from build123d import *

# Parameters (mm, degrees)
SKETCH3_R           = 46
SKETCH3_R_2         = 40
BOSS_EXTRUDE1_DEPTH = 215
SKETCH4_R           = 160
CUT_EXTRUDE1_DEPTH  = 900
CUT_EXTRUDE2_START  = -300
SKETCH5_R           = 40
CUT_EXTRUDE2_DEPTH  = 300
SKETCH6_R           = 67.5
SKETCH6_R_2         = 40
BOSS_EXTRUDE2_DEPTH = 15


with BuildPart() as part:
    # Sketch1 → Revolve1 (revolve)
    with BuildSketch(Plane.XY, mode=Mode.PRIVATE) as revolve1_sk:
        Polygon((0, 160), (0, 215), (40, 215), (40, 180), (1360, 180), (1390, 150), (1520, 150), (1520, 180), (1580, 180), (1580, 130), (1381.715728753, 130), (1351.715728753, 160), align=None)
    revolve(revolve1_sk.sketch.rotate(Axis((0, 0, 0), (1, 0, 0)), 90), axis=Axis((0, 0, 0), (1, 0, 0)))

    # Sketch3 → Boss-Extrude1 (add)
    with BuildSketch(Plane(origin=(0, 0, 0), x_dir=(1, 0, 0), z_dir=(0, 1, 0))):
        with Locations(Location((380, 0, 0), (0, 0, 90))):
            Circle(SKETCH3_R)
        with Locations(Location((380, 0, 0), (0, 0, 90))):
            Circle(SKETCH3_R_2, mode=Mode.SUBTRACT)
    extrude(amount=BOSS_EXTRUDE1_DEPTH)

    # Sketch4 → Cut-Extrude1 (cut)
    with BuildSketch(Plane.ZY):
        Circle(SKETCH4_R)
    extrude(amount=-CUT_EXTRUDE1_DEPTH, mode=Mode.SUBTRACT)

    # Sketch5 → Cut-Extrude2 (cut)
    with BuildSketch(Plane(origin=(0, 215, 0), x_dir=(1, 0, 0), z_dir=(0, 1, 0)).offset(CUT_EXTRUDE2_START)):
        with Locations(Location((380, 0, 0), (0, 0, 270))):
            Circle(SKETCH5_R)
    extrude(amount=CUT_EXTRUDE2_DEPTH, mode=Mode.SUBTRACT)

    # Sketch6 → Boss-Extrude2 (add)
    with BuildSketch(Plane(origin=(0, 215, 0), x_dir=(1, 0, 0), z_dir=(0, 1, 0))):
        with Locations(Location((380, 0, 0), (0, 0, 270))):
            Circle(SKETCH6_R)
        with Locations(Location((380, 0, 0), (0, 0, 270))):
            Circle(SKETCH6_R_2, mode=Mode.SUBTRACT)
    extrude(amount=BOSS_EXTRUDE2_DEPTH)


solid = part.part
Verification items for the finished model (mm, model axes). A direction names the side the tool comes from. Coordinates: 2 decimals unless noted, no trailing zeros. Write each loop counter-clockwise with the first axis right and the second up, starting at its lowest first coordinate (ties: lowest second). Pieces come first, ordered by that corner, then holes. Notation, with made-up numbers: M 60.5,-13.5 L 95.5,-13.5 A18 cw 95.5,13.5 Z; hole C 0.5,80.5 d5. An arc over 180 degrees is marked long. Use CSV: the item, a comma, the result in double quotes.
Q1. Mould release check, pull along X, two halves, no side actions. Record for faces 1 (the cylindrical face through (446.926, 222.395, -8.787)), 2 (the conical face through (1379.84, 117, 60.85)), 3 (the flat face through (1520, -134, 68)): pulls with the +X half, pulls with the -X half, needs draft (parallel to the pull), parting line crosses it, or undercut.
Computed values:
face 1,"parting line crosses it"
face 2,"pulls with the -X half"
face 3,"undercut"
Q2. Go/stop test with flat-tipped pins: P1, Ø8, axis at x = 1021, y = 131, coming from the -Z side; P2, Ø3, axis at x = 1267.5, z = 45, coming from the +Y side; P3, Ø5, axis at y = -127, z = -13, coming from the +X side; P4, Ø1.5, axis at x = 1024, z = -9.5, coming from the -Y side. Record where each tip stops, or that it passes through.
Computed values:
P1,"z = -127.56"
P2,"y = 174.66"
P3,"x = 1580"
P4,"y = -179.79"
Q3. Section check D-D, the plane x = 1253. Enter the section's corners in (y, z), and give its area (3 significant figures).
Computed values:
outline,"C 0,0 d360; hole C 0,0 d320"
area,"21,400 mm²"
Q4. Thickness scan on line 1 along X through (y, z) = (194.5, 0); line 2 along X through (y, z) = (226, 0); line 3 along Y through (x, z) = (1494, 0). Record the ranges inside material, lowest first. Write a range as [from, to].
Computed values:
line 1,"[0, 40], [334, 340], [420, 426]"
line 2,"[312.5, 340], [420, 447.5]"
line 3,"[-150, -130], [130, 150]"
Q5. Section check A-A, the plane y = 0. Enter the section's corners in (x, z), and give its area (3 significant figures).
Computed values:
outline,"M 0,-215 L 40,-215 L 40,-180 L 1360,-180 L 1390,-150 L 1520,-150 L 1520,-180 L 1580,-180 L 1580,-130 L 1381.72,-130 L 1351.72,-160 L 0,-160 Z; M 0,160 L 1351.72,160 L 1381.72,130 L 1580,130 L 1580,180 L 1520,180 L 1520,150 L 1390,150 L 1360,180 L 40,180 L 40,215 L 0,215 Z"
area,"70,100 mm²"
Q6. Section check C-C, the plane z = 0. State how many separate pieces and enclosed holes the cut face has, and give its area (3 significant figures).
Computed values:
separate pieces,"3"
enclosed holes,"0"
area,"69,700 mm²"
Q7. Set-up check for faces 4 (the conical face through (1388.54, -150.17, -19.72)), 5 (the cylindrical face through (1479.47, -39.048, 123.997)), 6 (the cylindrical face through (1550.42, 159.69, 83.06)): record each of +Z, -Z, +X, -X, +Y, -Y from which the full face is reachable in a straight line by a thin tool's end or side.
Computed values:
face 4,"none"
face 5,"+X, -X"
face 6,"+X"
Q8. Section check B-B, the plane x = 380. Enter the section's corners in (y, z).
Computed values:
outline,"M 154.92,-40 A160 cw long 154.92,40 L 230,40 L 230,67.5 L 215,67.5 L 215,46 L 174.02,46 A180 ccw long 174.02,-46 L 215,-46 L 215,-67.5 L 230,-67.5 L 230,-40 Z"
